The model under review builds one solid part; all positions refer to its coordinate system, in mm. Face numbers are marked on the shaded views. A direction names the side the tool comes from. Round coordinates to 2 decimals unless told otherwise and drop trailing zeros. Loops run counter-clockwise (first coordinate to the right, second up) from the corner with the lowest first, then second, coordinate; pieces in that order, holes last. Notation, with made-up numbers: M -28.75,34.5 L -0.75,34.5 A24 cw -0.75,55.5 Z; hole C -34,70.25 d6. An arc over 180 degrees is marked long. Return JSON: item names as keys, results as strings. Group by question number.
Q1. Consider section C-C (y = 2). Count the separate pieces of the cut face and the enclosed holes in it, and give its area (3 significant figures).
Q2. For the marked faces 4, 5 and 6, list the 3-axis set-ups (+Z, -Z, +X, -X, +Y, -Y) from which the entire face can be reached by the end or side of a thin tool; tool diameter is ignored.
Q3. To check wall thickness, follow line 1 along Z through (x, y) = (-87, 8); line 2 along Y through (x, z) = (-159, -17.5); line 3 along Z through (x, y) = (-117, 8). State the ranges of each line that lie inside material, in increasing order.
Q4. Consider section A-A (x = -87). State the section outline as (y, z) points, and give its area (3 significant figures).
Q5. Clearance check with flat-ended pins moving along their axes: pin 1 Ø4 at (y, z) = (6.5, 18) entering from +X; pin 2 Ø5 at (x, y) = (-93.5, 6) entering from +Z; pin 3 Ø5.5 at (x, z) = (-87, -17.5) entering from -Y; pin 4 Ø4 at (x, y) = (-81, 5) entering from -Z. State where each tip first meets the part, or that it passes through.
Q6. Draft analysis for pull direction X (two halves, no side actions). For the marked faces 1, 2 and 3, state which applies: pulls with the +X half, pulls with the -X half, needs draft (parallel to the pull), parting line crosses it, or undercut.
Q7. Consider section D-D (z = -17.5). State the section outline as (x, y) points.
Q8. Consider section B-B (z = 17.5). State the section outline as (x, y) points.
from build123d import *

# Parameters (mm, degrees)
SKETCH1_W             = 290
SKETCH1_H             = 45
BOSS_EXTRUDE1_DEPTH   = 10
SKETCH3_W             = 60
SKETCH3_H             = 10
CUT_EXTRUDE2_DEPTH    = 10
SKETCH4_W             = 45
SKETCH4_H             = 10
BOSS_EXTRUDE2_DEPTH   = 22
SKETCH6_R             = 5
CUT_EXTRUDE4_DEPTH    = 30
SKETCH7_W             = 80
SKETCH7_H             = 25
CUT_EXTRUDE5_DEPTH    = 27
SKETCH9_W             = 80
SKETCH9_H             = 45
CUT_EXTRUDE7_DEPTH    = 42
CUT_EXTRUDE8_DEPTH    = 20
SKETCH13_W            = 223.21076669
SKETCH13_H            = 10
CUT_EXTRUDE11_DEPTH   = 105
M5_TAPPED_HOLE1_D     = 4.2
M5_TAPPED_HOLE1_DEPTH = 12.4
M5_TAPPED_HOLE1_TIP   = 1.2618073
SKETCH19_W            = 55
SKETCH19_H            = 8
CUT_EXTRUDE13_DEPTH   = 169.805361289
SKETCH20_R            = 12.25
CUT_EXTRUDE14_DEPTH   = 174.245490562
M4_TAPPED_HOLE1_D     = 3.3
M4_TAPPED_HOLE1_DEPTH = 10.1
M4_TAPPED_HOLE1_TIP   = 0.991420021
CHAMFER1_SIZE         = 1
FILLET1_R             = 2
FILLET2_R             = 2


with BuildPart() as part:
    # Sketch1 → Boss-Extrude1 (new body)
    with BuildSketch(Plane(origin=(0, 0, 0), x_dir=(1, 0, 0), z_dir=(0, 1, 0))):
        Rectangle(SKETCH1_W, SKETCH1_H)
    extrude(amount=BOSS_EXTRUDE1_DEPTH)

    # Sketch3 → Cut-Extrude2 (cut)
    with BuildSketch(Plane(origin=(0, 10, 0), x_dir=(1, 0, 0), z_dir=(0, 1, 0))):
        with Locations((-105, 0.5)):
            Rectangle(SKETCH3_W, SKETCH3_H)
    extrude(amount=-CUT_EXTRUDE2_DEPTH, mode=Mode.SUBTRACT)

    # Sketch4 → Boss-Extrude2 (add)
    with BuildSketch(Plane.ZY.offset(145)):
        with Locations((0, 5)):
            Rectangle(SKETCH4_W, SKETCH4_H)
    extrude(amount=BOSS_EXTRUDE2_DEPTH)

    # Sketch6 → Cut-Extrude4 (cut)
    with BuildSketch(Plane(origin=(0, 10, 0), x_dir=(1, 0, 0), z_dir=(0, 1, 0))):
        with Locations(Location((-10, 0.5, 0), (0, 0, 270))):
            Circle(SKETCH6_R)
        with Locations(Location((-50, 0.5, 0), (0, 0, 270))):
            Circle(SKETCH6_R)
    extrude(amount=-CUT_EXTRUDE4_DEPTH, mode=Mode.SUBTRACT)

    # Sketch7 → Cut-Extrude5 (cut)
    with BuildSketch(Plane.XZ):
        with Locations((-30, -0.5)):
            Rectangle(SKETCH7_W, SKETCH7_H)
    extrude(amount=-CUT_EXTRUDE5_DEPTH, mode=Mode.SUBTRACT)

    # Sketch9 → Cut-Extrude7 (cut)
    with BuildSketch(Plane(origin=(0, 10, 0), x_dir=(1, 0, 0), z_dir=(0, 1, 0))):
        with Locations((-30, 0)):
            Rectangle(SKETCH9_W, SKETCH9_H)
    extrude(amount=-CUT_EXTRUDE7_DEPTH, mode=Mode.SUBTRACT)


with BuildPart() as cut_extrude7_piece_1:
    # of the separate pieces the step leaves, piece 1, a body of its own (cut_extrude7_pieces)
    add(part.part.solids().sort_by_distance((145, 0, -22.5))[0])

    # Sketch10 → Cut-Extrude8 (cut)
    with BuildSketch(Plane.XY.offset(22.5)):
        Polygon((145, 0), (145, 5), (130, 0), align=None)
    extrude(amount=-CUT_EXTRUDE8_DEPTH, mode=Mode.SUBTRACT)

    # Sketch13 → Cut-Extrude11 (cut)
    with BuildSketch(Plane.XY.offset(22.5)):
        with Locations((41.605383345, 5)):
            Rectangle(SKETCH13_W, SKETCH13_H)
    extrude(amount=-CUT_EXTRUDE11_DEPTH, mode=Mode.SUBTRACT)


with BuildPart() as cut_extrude7_piece_2:
    # of the separate pieces the step leaves, piece 2, a body of its own (cut_extrude7_pieces)
    add(part.part.solids().sort_by_distance((-70, 10, -22.5))[0])

    # M5 Tapped Hole1
    with Locations(Plane(origin=(-159, 5, -22.5), x_dir=(-1, 0, 0), z_dir=(0, 0, -1))):
        with Locations((0, 0), (-78, 0)):
            Hole(M5_TAPPED_HOLE1_D / 2, depth=M5_TAPPED_HOLE1_DEPTH)
            with Locations((0, 0, -(M5_TAPPED_HOLE1_DEPTH + M5_TAPPED_HOLE1_TIP / 2))):  # 118° drill point
                Cone(0, M5_TAPPED_HOLE1_D / 2, M5_TAPPED_HOLE1_TIP, mode=Mode.SUBTRACT)

    # Sketch19 → Cut-Extrude13 (cut, through all)
    with BuildSketch(Plane(origin=(0, 10, 0), x_dir=(1, 0, 0), z_dir=(0, 1, 0))):
        with Locations((-97.5, -18.5)):
            Rectangle(SKETCH19_W, SKETCH19_H)
    extrude(amount=-CUT_EXTRUDE13_DEPTH, mode=Mode.SUBTRACT)

    # Sketch20 → Cut-Extrude14 (cut, through all)
    with BuildSketch(Plane.XY.offset(22.5)):
        with Locations((-104.93, -5.3)):
            Circle(SKETCH20_R)
    extrude(amount=-CUT_EXTRUDE14_DEPTH, mode=Mode.SUBTRACT)

    # M4 Tapped Hole1
    with Locations(Plane(origin=(-152, 10, -17.5), x_dir=(0, 0, 1), z_dir=(0, 1, 0))):
        with Locations((0, 0), (0, 65), (35, 0)):
            Hole(M4_TAPPED_HOLE1_D / 2, depth=M4_TAPPED_HOLE1_DEPTH)
            with Locations((0, 0, -(M4_TAPPED_HOLE1_DEPTH + M4_TAPPED_HOLE1_TIP / 2))):  # 118° drill point
                Cone(0, M4_TAPPED_HOLE1_D / 2, M4_TAPPED_HOLE1_TIP, mode=Mode.SUBTRACT)

    # Chamfer1
    chamfer1_edges = [cut_extrude7_piece_2.edges().sort_by_distance(p)[0] for p in [
        (-167, 5, -22.5),
        (-167, 5, 22.5),
        (-70, 5, 14.5),
        (-125, 5, 22.5),
        (-70, 5, -22.5),
    ]]
    chamfer(chamfer1_edges, length=CHAMFER1_SIZE)

    # Fillet1
    fillet1_edges = [cut_extrude7_piece_2.edges().sort_by_distance(p)[0] for p in [
        (-125, 5, 14.5),
    ]]
    fillet(fillet1_edges, radius=FILLET1_R)

    # Fillet2
    fillet2_edges = [cut_extrude7_piece_2.edges().sort_by_distance(p)[0] for p in [
        (-75, 5, 4.5),
        (-135, 5, 4.5),
        (-135, 5, -5.5),
        (-75, 5, -5.5),
    ]]
    fillet(fillet2_edges, radius=FILLET2_R)


solid = cut_extrude7_piece_2.part
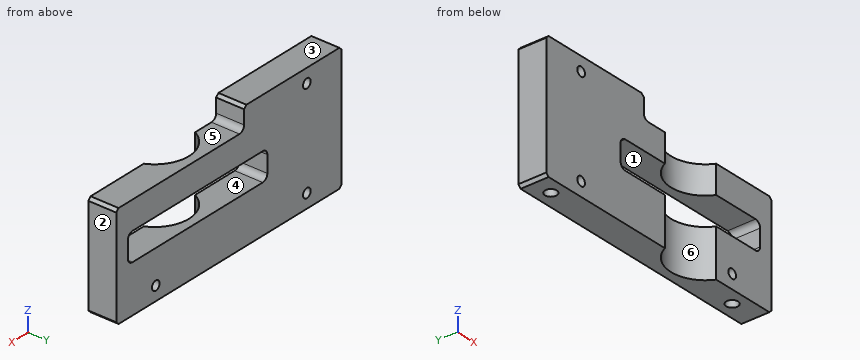
Values:
{
 "1": {"separate pieces": "2", "enclosed holes": "3", "area": "2,770 mm2"},
 "2": {"face 4": "+Y, -Y", "face 5": "+Z, +X, +Y, -Y", "face 6": "+Z, -Z, -Y"},
 "3": {"line 1": "z = -22.5 to -19.15, -15.85 to -5.5, 4.5 to 14.5", "line 2": "y = 0 to 2.9, 7.1 to 10", "line 3": "z = -22.5 to -5.5, 4.5 to 14.5"},
 "4": {"outline": "M 0,-22.5 L 10,-22.5 L 10,-19.15 L 0,-19.15 Z; M 0,-15.85 L 10,-15.85 L 10,-5.5 L 0,-5.5 Z; M 0,4.5 L 10,4.5 L 10,14.5 L 0,14.5 Z", "area": "237 mm2"},
 "5": {"pin 1": "stops at x = -124.94", "pin 2": "stops at z = 14.5", "pin 3": "stops at y = 0", "pin 4": "stops at z = -10.04"},
 "6": {"face 1": "undercut", "face 2": "pulls with the +X half", "face 3": "needs draft"},
 "7": {"outline": "M -167,0 L -153.65,0 L -153.65,10 L -167,10 Z; M -150.35,0 L -115.97,0 A12.25 cw -93.89,0 L -88.65,0 L -88.65,10 L -150.35,10 Z; M -85.35,0 L -70,0 L -70,10 L -85.35,10 Z; hole C -159,5 d4.2; hole C -81,5 d4.2"},
 "8": {"outline": "M -167,0 L -153.65,0 L -153.65,10 L -167,10 Z; M -150.35,0 L -125,0 L -125,10 L -150.35,10 Z"}
}
